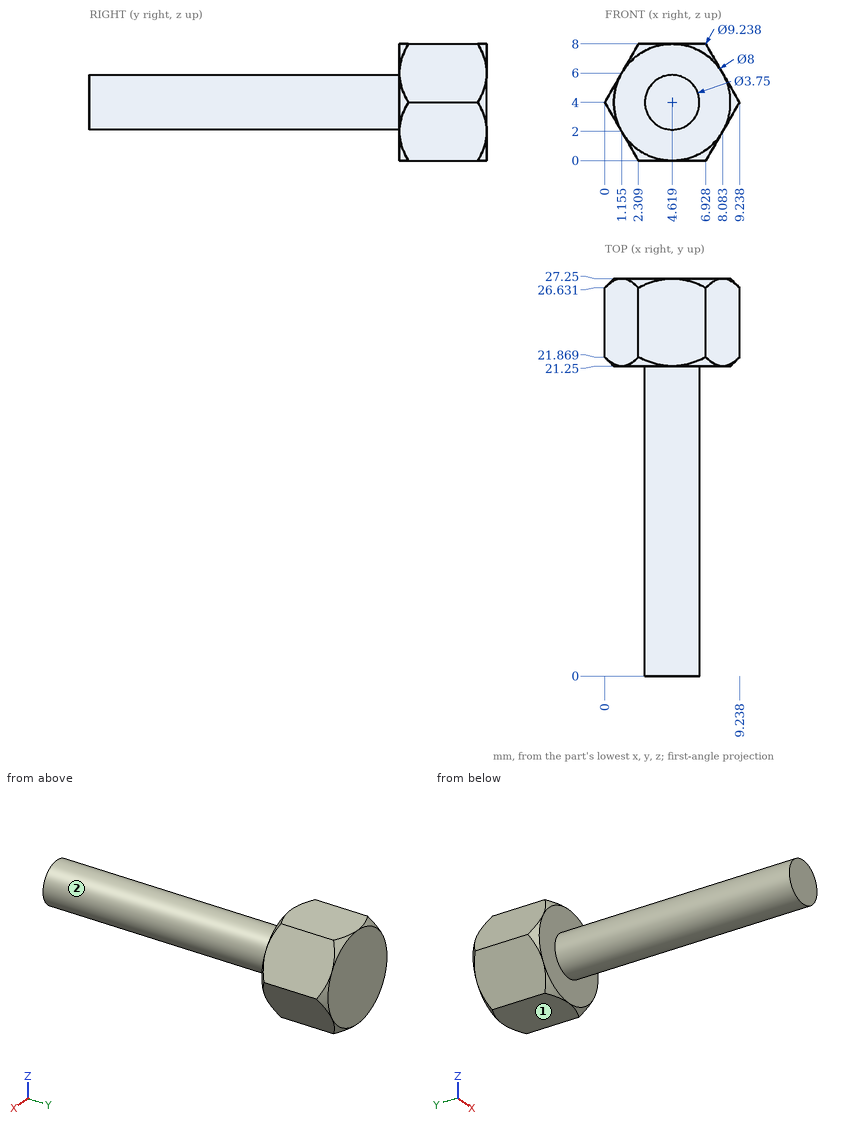
Geometry: see drawing. Coordinates: mm, zero at the bounding-box minimum. A direction names the side the tool comes from. Give positions to 0.01 mm unless a question says otherwise; leave off trailing zeros. One line per question, with ' | ' between items. Start each with the question number.
(1) Contact query for flat-ended pins moving along their axis: pin 1 (2 mm diameter, centred on y = 15, z = 1, fed in from -X); pin 2 (3 mm diameter, centred on y = 20, z = 5.5, fed in from +X). Output: stop coordinate, or through.
(2) Ray query, line 1 (X direction, y = 25.5, z = 2) (1 decimal); line 2 (Y direction, x = 7.5, z = 2.75); line 3 (Z direction, x = 4.5, y = 19.5). Return the intervals inside material, ascending. Write a range as from..to.
(3) Reachability of the marked faces 1 and 2 from +Z, -Z, +X, -X, +Y, -Y: full face, straight path, thin tool, end or side. Return the list, or none.
The answers:
1) pin 1: through | pin 2: x = 8.66
2) line 1: 1.2..8.1 | line 2: 21.25..27.25 | line 3: 2.13..5.87
3) face 1: -Z, +X, -X, +Y, -Y | face 2: -Y
